Here's how the part is built. I have some questions about the finished solid (model axes, mm). Face numbers are marked on the shaded views. A direction names the side the tool comes from. Give positions to 0.01 mm unless a question says otherwise; leave off trailing zeros. One line per item, written item: value. Start each with the question number.
1) We'd pull the mould along Y, two halves only. Please class the marked faces 1, 2, 3 and 4: +Y half, -Y half, draft (parallel to the pull), parting line (faces both ways), or undercut.
2) Imagine slicing it at A-A on z = -51. Count the separate pieces of the cut face and the enclosed holes in it, plus the area to 3 significant figures.
3) On a 3-axis mill with a long thin cutter (end or side, diameter ignored), from which of +Z, -Z, +X, -X, +Y, -Y can I reach the whole of each face in a straight line? I mean the marked faces 5, 6, 7, 8 and 9. Say none if no direction works.
4) Please list where these lines run through material, in increasing order: L1, parallel to Y at x = -14.5, z = -19; L2, parallel to X at y = -14.5, z = -56.5; L3, parallel to Y at x = -13.5, z = -20.5. Write a range as [from, to].
5) I'm going to push flat-ended pins straight in: P1, Ø6, axis at x = 15, y = -15, coming from the -Z side; P2, Ø2, axis at x = 8.5, y = -8, coming from the +Z side; P3, Ø8, axis at y = -7, z = -55, coming from the -X side; P4, Ø10, axis at x = -15.5, y = 11.5, coming from the -Z side. Where does each tip first touch, or does it pass through?
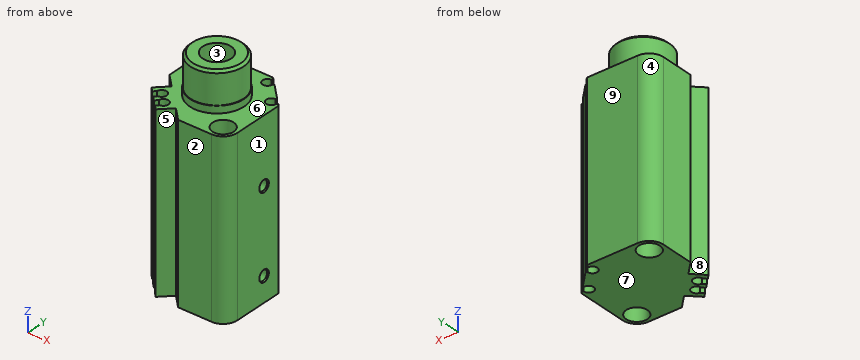
from build123d import *

# Parameters (mm, degrees)
EXTRUDE_1_DEPTH = 73


with BuildPart() as part:
    # 草图1 → 凸台-拉伸1 (new body)
    with BuildSketch(Plane.XY):
        with BuildLine():
            Line((-20, 14), (-20, -0.223253942))
            Line((-20, -0.223253942), (-14.919953083, -5.303300859))
            Line((-14.919953083, -5.303300859), (-19.657568517, -10.040916293))
            Line((-19.657568517, -10.040916293), (-17.960512242, -11.737972568))
            Line((-17.960512242, -11.737972568), (-16.828035921, -10.605496246))
            ThreePointArc((-16.828035921, -10.605496246), (-13.205219139, -9.245421164), (-14.565294221, -12.868237946))
            Line((-14.565294221, -12.868237946), (-15.697770542, -14.000714267))
            Line((-15.697770542, -14.000714267), (-14.000714267, -15.697770542))
            Line((-14.000714267, -15.697770542), (-12.868237946, -14.565294221))
            ThreePointArc((-12.868237946, -14.565294221), (-9.245421164, -13.205219139), (-10.605496246, -16.828035921))
            Line((-10.605496246, -16.828035921), (-11.737972568, -17.960512242))
            Line((-11.737972568, -17.960512242), (-10.040916293, -19.657568517))
            Line((-10.040916293, -19.657568517), (-5.303300859, -14.919953083))
            Line((-5.303300859, -14.919953083), (-0.223253942, -20))
            Line((-0.223253942, -20), (14, -20))
            ThreePointArc((14, -20), (18.242640687, -18.242640687), (20, -14))
            Line((20, -14), (20, 7.577164466))
            Line((20, 7.577164466), (19.091883092, 8.485281374))
            Line((19.091883092, 8.485281374), (18.671295499, 8.064693782))
            ThreePointArc((18.671295499, 8.064693782), (15.04369677, 6.558415396), (16.549975156, 10.186014125))
            Line((16.549975156, 10.186014125), (16.970562748, 10.606601718))
            Line((16.970562748, 10.606601718), (10.606601718, 16.970562748))
            Line((10.606601718, 16.970562748), (10.186014125, 16.549975156))
            ThreePointArc((10.186014125, 16.549975156), (6.558415396, 15.04369677), (8.064693782, 18.671295499))
            Line((8.064693782, 18.671295499), (8.485281374, 19.091883092))
            Line((8.485281374, 19.091883092), (7.577164466, 20))
            Line((7.577164466, 20), (-14, 20))
            ThreePointArc((-14, 20), (-18.242640687, 18.242640687), (-20, 14))
        make_face()
    extrude(amount=-EXTRUDE_1_DEPTH)

    # 草图2 → 切除-旋转1 (revolve, cut)
    with BuildSketch(Plane(origin=(0, 0, 0), x_dir=(0.7071067811865476, -0.7071067811865475, 0), z_dir=(0.7071067811865475, 0.7071067811865476, 0)), mode=Mode.PRIVATE) as cut_revolve_1_sk:
        Polygon((20, 73), (24.5, 73), (24.5, 66), (23, 66), (22.4585, 65.4585), (22.4585, 56), (22.75, 56), (22.75, 17), (22.4585, 17), (22.4585, 7.5415), (23, 7), (24.5, 7), (24.5, 0), (20, 0), align=None)
    revolve(cut_revolve_1_sk.sketch.rotate(Axis((14.142135624, -14.142135624, 0), (0, 0, -1)), 135), axis=Axis((14.142135624, -14.142135624, 0), (0, 0, -1)), mode=Mode.SUBTRACT)

    # 草图3 → 切除-旋转2 (revolve, cut)
    with BuildSketch(Plane(origin=(0, 0, 0), x_dir=(0.7071067811865476, -0.7071067811865475, 0), z_dir=(0.7071067811865475, 0.7071067811865476, 0)), mode=Mode.PRIVATE) as cut_revolve_2_sk:
        Polygon((-20, 73), (-15.5, 73), (-15.5, 66), (-17, 66), (-17.5415, 65.4585), (-17.5415, 56), (-17.25, 56), (-17.25, 17), (-17.5415, 17), (-17.5415, 7.5415), (-17, 7), (-15.5, 7), (-15.5, 0), (-20, 0), align=None)
    revolve(cut_revolve_2_sk.sketch.rotate(Axis((-14.142135624, 14.142135624, 0), (0, 0, -1)), 135), axis=Axis((-14.142135624, 14.142135624, 0), (0, 0, -1)), mode=Mode.SUBTRACT)

    # 草图4 → 旋转1 (revolve)
    with BuildSketch(Plane(origin=(0, 0, 0), x_dir=(1, 0, 0), z_dir=(0, 1, 0)), mode=Mode.PRIVATE) as revolve_1_sk:
        Polygon((0, 0), (11.5, 0), (11.5, -3), (11.25, -3), (11.25, -15.5), (10.25, -16.5), (0, -16.5), align=None)
    revolve(revolve_1_sk.sketch.rotate(Axis((0, 0, 16.5), (0, 0, -1)), 180), axis=Axis((0, 0, 16.5), (0, 0, -1)))

    # 草图5 → 切除-旋转3 (revolve, cut)
    with BuildSketch(Plane(origin=(0, 0, 0), x_dir=(1, 0, 0), z_dir=(0, 1, 0)), mode=Mode.PRIVATE) as cut_revolve_3_sk:
        Polygon((0, 54.5), (12.5, 54.5), (12.5, 20), (6, 20), (6, -16.5), (0, -16.5), align=None)
    revolve(cut_revolve_3_sk.sketch.rotate(Axis((0, 0, 16.5), (0, 0, -1)), 180), axis=Axis((0, 0, 16.5), (0, 0, -1)), mode=Mode.SUBTRACT)

    # 草图6 → 切除-旋转4 (revolve, cut)
    with BuildSketch(Plane(origin=(0, 0, 0), x_dir=(1, 0, 0), z_dir=(0, 1, 0)), mode=Mode.PRIVATE) as cut_revolve_4_sk:
        Polygon((20, 27.5), (20, 25), (19.567, 25.433), (15, 25.433), (13.806616994, 27.5), align=None)
    revolve(cut_revolve_4_sk.sketch.rotate(Axis((13.806616994, 0, -27.5), (1, 0, 0)), 180), axis=Axis((13.806616994, 0, -27.5), (1, 0, 0)), mode=Mode.SUBTRACT)

    # 草图7 → 切除-旋转5 (revolve, cut)
    with BuildSketch(Plane(origin=(0, 0, 0), x_dir=(1, 0, 0), z_dir=(0, 1, 0)), mode=Mode.PRIVATE) as cut_revolve_5_sk:
        Polygon((20, 62.5), (20, 60), (19.567, 60.433), (15, 60.433), (13.806616994, 62.5), align=None)
    revolve(cut_revolve_5_sk.sketch.rotate(Axis((13.806616994, 0, -62.5), (1, 0, 0)), 180), axis=Axis((13.806616994, 0, -62.5), (1, 0, 0)), mode=Mode.SUBTRACT)


solid = part.part
Numbers:
1. face 1: draft
1. face 2: -Y half
1. face 3: undercut
1. face 4: +Y half
2. separate pieces: 1
2. enclosed holes: 3
2. area: 800 mm^2
3. face 5: +Z, -Z, -Y
3. face 6: +Z
3. face 7: -Z, +X, -X, +Y, -Y
3. face 8: +Z, -Z, -X
3. face 9: +Z, -Z, +X, -X, +Y
4. L1: [-15.2, -12.86], [-8.63, 11.42], [16.87, 19.98]
4. L2: [-15.2, -12.86], [-8.63, 11.71], [16.57, 19.98]
4. L3: [-15.2, -12.5], [-9, 11.47], [16.82, 20]
5. P1: z = -66
5. P2: z = 16.08
5. P3: x = -19.66
5. P4: z = -73
